Design review of the part built by this model. Coordinates are the model's own, in mm. A direction names the side the tool comes from. Give positions to 0.01 mm unless a question says otherwise; leave off trailing zeros. Write each loop counter-clockwise with the first axis right and the second up, starting at its lowest first coordinate (ties: lowest second). Pieces come first, ordered by that corner, then holes. Notation, with made-up numbers: M 88.25,87 L 147.25,87 A8 cw 147.25,96 Z; hole C 35,55.5 d8. An arc over 180 degrees is marked long. Use one line per item in the form item = value. Start each with the question number.
from build123d import *

# Parameters (mm, degrees)
SHAFT_BASE_30_SKETCH_R     = 15
SHAFT_BASE_30_DEPTH        = 45
SHAFT_STEP_2_SKETCH_R      = 10
SHAFT_STEP_2_DEPTH         = 16
SHAFT_TIP_SKETCH_R         = 4
SHAFT_TIP_DEPTH            = 19
CONE_SMALL_END_36_SKETCH_R = 18
CONE_BASE_100_SKETCH_R     = 50
GROOVE_SWEEP_CUT_PROFILE_R = 2.5


with BuildPart() as part:
    # Shaft Base Ø30 Sketch → Shaft Base Ø30 (new body)
    with BuildSketch(Plane.XY):
        with Locations(Location((0, 0, 0), (0, 0, 180))):
            Circle(SHAFT_BASE_30_SKETCH_R)
    extrude(amount=SHAFT_BASE_30_DEPTH)

    # Shaft Step 2 Sketch → Shaft Step 2 (add)
    with BuildSketch(Plane.XY.offset(45)):
        Circle(SHAFT_STEP_2_SKETCH_R)
    extrude(amount=SHAFT_STEP_2_DEPTH)

    # Shaft Tip Sketch → Shaft Tip (add)
    with BuildSketch(Plane.XY.offset(61)):
        Circle(SHAFT_TIP_SKETCH_R)
    extrude(amount=SHAFT_TIP_DEPTH)

    # Cone Small End Ø36 Sketch → Conical Body section 0
    with BuildSketch(Plane(origin=(0, 0, -85), x_dir=(-1, 0, 0), z_dir=(0, 0, -1))):
        Circle(CONE_SMALL_END_36_SKETCH_R)
    # Cone Base Ø100 Sketch → Conical Body section 1
    with BuildSketch(Plane(origin=(0, 0, 0), x_dir=(-1, 0, 0), z_dir=(0, 0, -1))):
        Circle(CONE_BASE_100_SKETCH_R)
    loft()

    # Groove Sweep Cut: sweep along a path in Groove Path
    with BuildLine(Plane(origin=(0, 0, -72.5), x_dir=(-1, 0, 0), z_dir=(0, 0, -1))) as groove_sweep_cut_path:
        CenterArc((0, 0), 22.673462662, 0, 360)
    # Groove Sweep Cut profile (on start of the path) → Groove Sweep Cut (sweep, cut)
    with BuildSketch(Plane(origin=(-22.673462662, 0, -72.5), x_dir=(0, 0, 1), z_dir=(0, 1, 0))):
        Circle(GROOVE_SWEEP_CUT_PROFILE_R)
    sweep(path=groove_sweep_cut_path.line, mode=Mode.SUBTRACT)


solid = part.part
1. We need section C-C (z = -29). State the section outline as (x, y) points, and give its area (3 significant figures).
2. We need section B-B (z = 30). State the section outline as (x, y) points.
3. To check wall thickness, follow L1, parallel to Z at x = -14, y = -10; L2, parallel to Z at x = -10, y = 18; L3, parallel to Z at x = -20, y = -7. State the ranges of each line that lie inside material, in increasing order.
4. We need section A-A (x = 0). State the section outline as (y, z) points.
5. Clearance check with flat-ended pins moving along their axes: pin 1 Ø1.5 at (y, z) = (18, -11.5) entering from +X; pin 2 Ø12 at (y, z) = (-18, -68) entering from -X; pin 3 Ø5 at (x, z) = (14, 58.5) entering from -Y; pin 4 Ø2 at (y, z) = (35.5, -2.5) entering from -X. State where each tip first meets the part, or that it passes through.
6. For faces 1 (the cylindrical face through (-2.17, -9.76, 52.89)), 2 (the flat face through (0, 0, -85)), list the 3-axis set-ups (+Z, -Z, +X, -X, +Y, -Y) from which the entire face can be reached by the end or side of a thin tool; tool diameter is ignored.
Answer block:
q1.outline = C 0,0 d78.16
q1.area = 4,800 mm^2
q2.outline = C 0,0 d30
q3.L1 = -85 to 0
q3.L2 = -78.12 to -73.88, -71.12 to 0
q3.L3 = -76.53 to -74.51, -70.49 to 0
q4.outline = M -50,0 L -23.58,-70.17 A2.5 cw long -21.82,-74.85 L -18,-85 L 18,-85 L 21.82,-74.85 A2.5 cw long 23.58,-70.17 L 50,0 L 15,0 L 15,45 L 10,45 L 10,61 L 4,61 L 4,80 L -4,80 L -4,61 L -10,61 L -10,45 L -15,45 L -15,0 Z
q5.pin_1 = 42.41
q5.pin_2 = -22.12
q5.pin_3 = through
q5.pin_4 = -35.01
q6.face_1 = +Z
q6.face_2 = -Z, +X, -X, +Y, -Y
